```python
from build123d import *


with BuildPart() as part:
    # Sketch1 → Revolve1 (revolve)
    with BuildSketch(Plane.XY, mode=Mode.PRIVATE) as revolve1_sk:
        with BuildLine():
            Line((0, 0), (25.5, 0))
            Line((25.5, 0), (25.5, 10))
            Line((25.5, 10), (17, 10))
            Line((17, 10), (17, 73.542486889))
            ThreePointArc((17, 73.542486889), (19.583426132, 87.684622513), (27, 100))
            Line((27, 100), (27, 120))
            Line((27, 120), (17, 130))
            Line((17, 130), (7.997028415, 460.218028737))
            ThreePointArc((7.997028415, 460.218028737), (5.57923696, 465.733420876), (0, 468))
            Line((0, 468), (0, 0))
        make_face()
    revolve(revolve1_sk.sketch.rotate(Axis((0, 0, 0), (0, -1, 0)), 90), axis=Axis((0, 0, 0), (0, -1, 0)))


solid = part.part
```
The listing builds one solid part. Answer for the finished solid, in the listing's coordinates (mm). A direction names the side the tool comes from. Coordinates: 2 decimals unless noted, no trailing zeros. Write each loop counter-clockwise with the first axis right and the second up, starting at its lowest first coordinate (ties: lowest second). Pieces come first, ordered by that corner, then holes. Notation, with made-up numbers: (-37.75, 46.25) -> (9.25, 46.25) arc R20 cw to (9.25, 71.25) -> close; hole circle Ø5 at (77, 42.25). An arc over 180 degrees is marked (long way). Write each question's results on one line, items separated by ' | '. Start each with the question number.
1) A tool of negligible diameter and unlimited length cuts with its end or side. For faces 1 (the cylindrical face through (15.516, 5.07, -20.236)), 2 (the cylindrical face through (-16.855, 42.216, -2.213)), 3 (the flat face through (0, 0, 0)), from which of +Z, -Z, +X, -X, +Y, -Y can it reach the whole face along a straight path? Write none if from no direction.
2) A cutting plane is placed at C-C (y = 145). Determine the outline of the cut face in (x, z), then the cut area to 3 significant figures.
3) Flat-ended cylindrical pins translate along their axes: pin 1 Ø1 at (y, z) = (167.5, 12.5) entering from -X; pin 2 Ø1.5 at (x, y) = (15, 151.5) entering from -Z; pin 3 Ø10 at (x, y) = (11, 347.5) entering from +Z. Find the tip coordinate at first contact, or state that the pin passes through.
4) For a pull along Y with two mould halves and no side action, classify faces 4 (the flat face through (17, 10, 5)), 5 (the cylindrical face through (26.36, 110.14, -5.85)), 6 (the conical face through (-3.74, 297.42, 11.86)) as +Y half, -Y half, draft (parallel to the pull), parting line (faces both ways), or undercut.
5) A cutting plane is placed at D-D (y = 411). Determine the outline of the cut face in (x, z).
6) Straight lines are drawn through the part: probe 1 along Y at (x, z) = (-10, -18); probe 2 along Y at (x, z) = (6, 23.5); probe 3 along X at (y, z) = (68.5, -8.5). For each, find the intervals that lie inside material, in ascending order.
7) A cutting plane is placed at A-A (z = 0). Determine the outline of the cut face in (x, y), then the cut area to 3 significant figures.
8) A cutting plane is placed at B-B (x = 0). Determine the outline of the cut face in (y, z).
Values follow:
1) face 1: -Y | face 2: none | face 3: +Z, -Z, +X, -X, -Y
2) outline: circle Ø33.18 at (0, 0) | area: 865 mm²
3) pin 1: x = -10.55 | pin 2: z = -8.15 | pin 3: z = 9.31
4) face 4: undercut | face 5: draft | face 6: +Y half
5) outline: circle Ø18.68 at (0, 0)
6) probe 1: 0 to 10, 90.11 to 126.41 | probe 2: 0 to 10, 96.51 to 122.75 | probe 3: -14.72 to 14.72
7) outline: (-27, 100) arc R40 cw to (-17, 73.54) -> (-17, 10) -> (-25.5, 10) -> (-25.5, 0) -> (25.5, 0) -> (25.5, 10) -> (17, 10) -> (17, 73.54) arc R40 cw to (27, 100) -> (27, 120) -> (17, 130) -> (8, 460.22) arc R8 ccw to (-8, 460.22) -> (-17, 130) -> (-27, 120) -> close | area: 13,600 mm²
8) outline: (0, -25.5) -> (10, -25.5) -> (10, -17) -> (73.54, -17) arc R40 cw to (100, -27) -> (120, -27) -> (130, -17) -> (460.22, -8) arc R8 ccw to (460.22, 8) -> (130, 17) -> (120, 27) -> (100, 27) arc R40 cw to (73.54, 17) -> (10, 17) -> (10, 25.5) -> (0, 25.5) -> close
